from build123d import *

# Parameters (mm, degrees)
SKETCH_1_W                   = 86
SKETCH_1_H                   = 58
SKETCH_1_R                   = 16
SKETCH_1_R_2                 = 2.25
EXTRUDE_1_DEPTH              = 5
HOLE_WIZARD_M3_1_D           = 2.5
HOLE_WIZARD_M4_1_D           = 3.3
MIRROR_2_COPY_1_D            = 3.3
CUT_EXTRUDE_1_DEPTH          = 53.820450585
CHAMFER_1_SIZE               = 1
SKETCH_10_W                  = 216.550460162
SKETCH_10_H                  = 17.046792279
CUT_EXTRUDE_4_DEPTH          = 73.374028491
SKETCH_11_R                  = 19.5
CUT_EXTRUDE_5_DEPTH          = 2.6
SKETCH_13_R                  = 1.350406535
CUT_EXTRUDE_6_DEPTH          = 10
HOLE_WIZARD_M4_3_D           = 3.3
HOLE_WIZARD_M4_3_DEPTH       = 11.5
HOLE_WIZARD_M4_3_CSINK_D     = 4.05
HOLE_WIZARD_M4_3_CSINK_ANGLE = 90
HOLE_WIZARD_M4_3_TIP         = 0.991420021


with BuildPart() as part:
    # 草图1 → 凸台-拉伸1 (new, symmetric)
    with BuildSketch(Plane.XY):
        Rectangle(SKETCH_1_W, SKETCH_1_H)
        Circle(SKETCH_1_R, mode=Mode.SUBTRACT)
        with Locations((-39, 24)):
            Circle(SKETCH_1_R_2, mode=Mode.SUBTRACT)
        with Locations(Location((39, 24, 0), (0, 0, 180))):
            Circle(SKETCH_1_R_2, mode=Mode.SUBTRACT)
        with Locations((39, -24)):
            Circle(SKETCH_1_R_2, mode=Mode.SUBTRACT)
        with Locations(Location((-39, -24, 0), (0, 0, 180))):
            Circle(SKETCH_1_R_2, mode=Mode.SUBTRACT)
    extrude(amount=EXTRUDE_1_DEPTH, both=True)

    # M3 螺纹孔1 (through all)
    with Locations(Plane.XY.offset(5)):
        with Locations((-38.5, 15), (-19.5, 15)):
            Hole(HOLE_WIZARD_M3_1_D / 2)

    # M4 螺纹孔1 (through all)
    with Locations(Plane.XY.offset(5)):
        with Locations((-23.57, 23.57)):
            hole_wizard_m4_1 = Hole(HOLE_WIZARD_M4_1_D / 2)

    # 镜向1: M4 螺纹孔1 across plane
    add(hole_wizard_m4_1.mirror(Plane.ZX), mode=Mode.SUBTRACT)

    # 镜向2: M4 螺纹孔1 across plane
    add(hole_wizard_m4_1.mirror(Plane(origin=(0, 0, 0), x_dir=(0, 0, 1), z_dir=(1, 0, 0))), mode=Mode.SUBTRACT)

    # 镜向2 copy 1 (through all)
    with Locations(Plane(origin=(0, 0, 5), x_dir=(-1, 0, 0), z_dir=(0, 0, 1))):
        with Locations((-23.57, 23.57)):
            Hole(MIRROR_2_COPY_1_D / 2)

    # 草图7 → 切除-拉伸1 (cut, through all)
    with BuildSketch(Plane.XY.offset(5)):
        with BuildLine():
            Line((-33, -29), (-33, -26))
            ThreePointArc((-33, -26), (-31, -24), (-29, -26))
            Line((-29, -26), (-29, -29))
            ThreePointArc((-29, -29), (-31, -31), (-33, -29))
        make_face()
    extrude(amount=-CUT_EXTRUDE_1_DEPTH, mode=Mode.SUBTRACT)

    # 倒角1
    chamfer_1_edges = [part.edges().sort_by_distance(p)[0] for p in [
        (43, -29, 0),
        (-43, -29, 0),
        (-43, 29, 0),
        (43, 29, 0),
    ]]
    chamfer(chamfer_1_edges, length=CHAMFER_1_SIZE)

    # 草图10 → 切除-拉伸4 (cut, through all)
    with BuildSketch(Plane(origin=(0, 29, 0), x_dir=(1, 0, 0), z_dir=(0, 1, 0))):
        with Locations((51.936518235, 8.52339614)):
            Rectangle(SKETCH_10_W, SKETCH_10_H)
    extrude(amount=-CUT_EXTRUDE_4_DEPTH, mode=Mode.SUBTRACT)

    # 草图11 → 切除-拉伸5 (cut)
    with BuildSketch(Plane(origin=(0, 0, 0), x_dir=(-1, 0, 0), z_dir=(0, 0, -1))):
        Circle(SKETCH_11_R)
    extrude(amount=-CUT_EXTRUDE_5_DEPTH, mode=Mode.SUBTRACT)

    # 草图13 → 切除-拉伸6 (cut)
    with BuildSketch(Plane.XY.offset(5)):
        with Locations((29, -11)):
            Circle(SKETCH_13_R)
    extrude(amount=-CUT_EXTRUDE_6_DEPTH, mode=Mode.SUBTRACT)

    # M4 螺纹孔3
    with Locations(Plane(origin=(29, -11, 5), x_dir=(1, 0, 0), z_dir=(0, 0, 1))):
        with Locations((0, 0)):
            CounterSinkHole(HOLE_WIZARD_M4_3_D / 2, HOLE_WIZARD_M4_3_CSINK_D / 2, depth=HOLE_WIZARD_M4_3_DEPTH, counter_sink_angle=HOLE_WIZARD_M4_3_CSINK_ANGLE)
            with Locations((0, 0, -(HOLE_WIZARD_M4_3_DEPTH + HOLE_WIZARD_M4_3_TIP / 2))):  # 118° drill point
                Cone(0, HOLE_WIZARD_M4_3_D / 2, HOLE_WIZARD_M4_3_TIP, mode=Mode.SUBTRACT)


solid = part.part
The listing builds one solid part. Answer for the finished solid, in the listing's coordinates (mm). A direction names the side the tool comes from. Round coordinates to 2 decimals unless told otherwise and drop trailing zeros. Write each loop counter-clockwise with the first axis right and the second up, starting at its lowest first coordinate (ties: lowest second). Pieces come first, ordered by that corner, then holes. Notation, with made-up numbers: (-30, 81) - (-7, 81) arc R23 cw to (-7, 99) - close; hole circle Ø4 at (18.5, 52.25). An arc over 180 degrees is marked (long way). Use a Markdown table: item, result. Add a question column.
1. For a pull along X with two mould halves and no side action, classify faces 4 (the face through (23.21, 21.96, 2.46)), 5 (the face through (-10, 13, 5)), 6 (the face through (-43, 0, 3)) as +X half, -X half, draft (parallel to the pull), parting line (faces both ways), or undercut.
2. Consider line 1 (Y direction, x = 23.57, z = 3.45); line 2 (Y direction, x = 39, z = 2.7); line 3 (X direction, y = -25, z = 1.95). Determine where each line is inside the solid, lowest interval first.
3. The part is cut by section B-B (x = 0). Write down the section's boundary in (y, z).
4. The part is cut by section D-D (y = -7). Write down the section's boundary in (x, z), and give its area (3 significant figures).
5. A tool of negligible diameter and unlimited length cuts with its end or side. For faces 1 (the face through (39.488, 26.196, 2.465)), 2 (the face through (-33, -28, 3)), 3 (the face through (-3, 16, 2.6)), from which of +Z, -Z, +X, -X, +Y, -Y can it reach the whole face along a straight path? Write none if from no direction.
6. A flat-ended cylindrical pin translates along its axis: P1, Ø4, axis at x = 29, y = -11, coming from the +Z side (3 decimals). Find the tip coordinate at first contact, or state that the pin passes through.
7. The part is cut by section C-C (z = 3.65). Give the number of separate pieces and of enclosed holes in the cut face, and give its area (3 significant figures).
8. The part is cut by section A-A (x = 39). Write down the section's boundary in (y, z), and give its area (3 significant figures).
Reported:
| question | item | result |
|---|---|---|
| 1 | face 4 | undercut |
| 1 | face 5 | draft |
| 1 | face 6 | -X half |
| 2 | line 1 | -29 to -25.22, -21.92 to 21.92, 25.22 to 29 |
| 2 | line 2 | -29 to -26.25, -21.75 to 21.75, 26.25 to 29 |
| 2 | line 3 | -43 to -41.02, -36.98 to -32.73, -29.27 to -24.39, -22.75 to 22.75, 24.39 to 36.98, 41.02 to 43 |
| 3 | outline | (-29, 0) - (-19.5, 0) - (-19.5, 2.6) - (-16, 2.6) - (-16, 5) - (-29, 5) - close; (16, 2.6) - (19.5, 2.6) - (19.5, 0) - (29, 0) - (29, 5) - (16, 5) - close |
| 4 | outline | (-43, 0) - (-18.2, 0) - (-18.2, 2.6) - (-14.39, 2.6) - (-14.39, 5) - (-43, 5) - close; (14.39, 2.6) - (18.2, 2.6) - (18.2, 0) - (43, 0) - (43, 5) - (14.39, 5) - close |
| 4 | area | 266 mm^2 |
| 5 | face 1 | +Z, -Z |
| 5 | face 2 | +Z, -Z, -Y |
| 5 | face 3 | -Z |
| 6 | P1 | z = 4.975 |
| 7 | separate pieces | 1 |
| 7 | enclosed holes | 12 |
| 7 | area | 4,050 mm^2 |
| 8 | outline | (-29, 0) - (-26.25, 0) - (-26.25, 5) - (-29, 5) - close; (-21.75, 0) - (21.75, 0) - (21.75, 5) - (-21.75, 5) - close; (26.25, 0) - (29, 0) - (29, 5) - (26.25, 5) - close |
| 8 | area | 245 mm^2 |
